The figure shows three views and two pictorial views of one solid part (mm, origin at its lowest corner). Answer the questions. Round coordinates to 2 decimals unless told otherwise and drop trailing zeros. Write each loop counter-clockwise with the first axis right and the second up, starting at its lowest first coordinate (ties: lowest second). Pieces come first, ordered by that corner, then holes. Notation, with made-up numbers: M -26,43 L 12,43 A20 cw 12,78 Z; hole C 38.5,42 d6. An arc over 180 degrees is marked long. Answer in a Markdown table with one row per item.
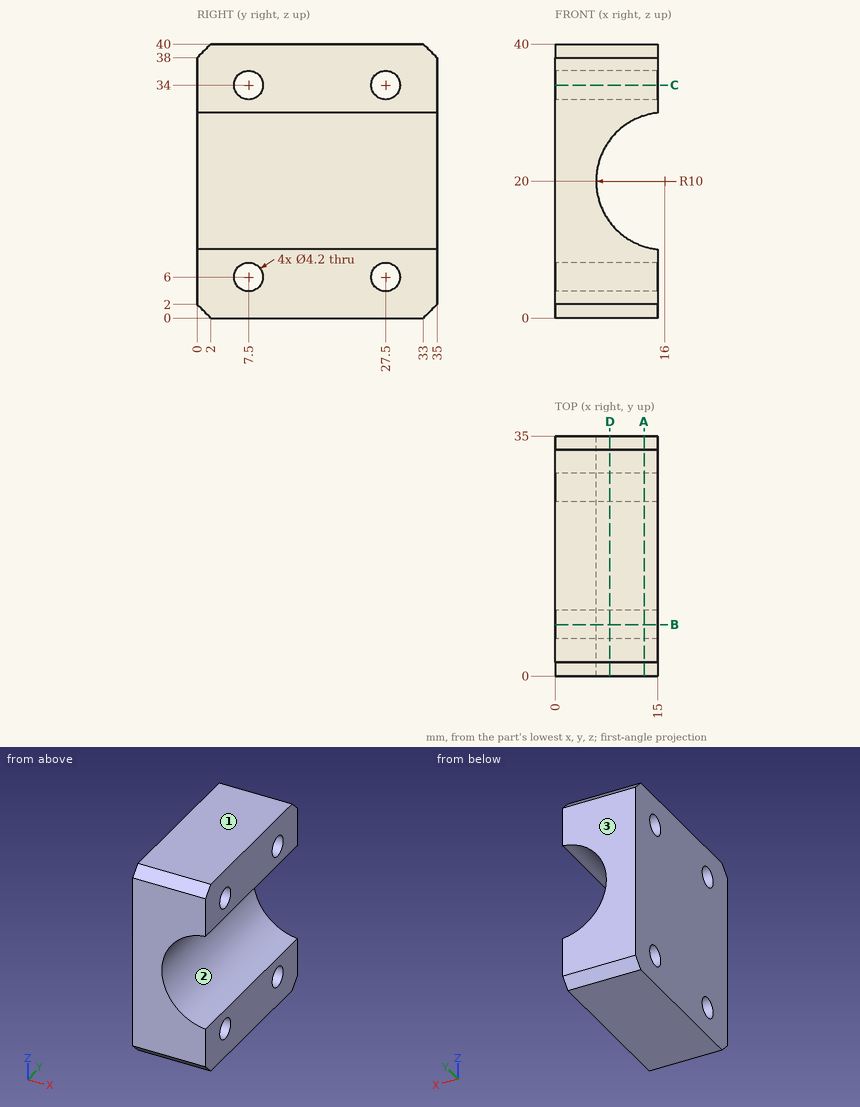
1. Given pin 1 (2 mm diameter, centred on y = 18, z = 26, fed in from +X), flat-ended and moving along its own axis, determine where the tip first touches the part or whether it passes through.
Calculated:
| item | result |
|---|---|
| pin 1 | stops at x = 8.86 |
2. The part is cut by section B-B (y = 7.5). Determine the outline of the cut face in (x, z), plus the area to 3 significant figures.
Calculated:
| item | result |
|---|---|
| outline | M 0,0 L 15,0 L 15,3.9 L 0,3.9 Z; M 0,8.1 L 15,8.1 L 15,10.05 A10 cw 15,29.95 L 15,31.9 L 0,31.9 Z; M 0,36.1 L 15,36.1 L 15,40 L 0,40 Z |
| area | 337 mm² |
3. The part is cut by section D-D (x = 8). Determine the outline of the cut face in (y, z), plus the area to 3 significant figures.
Calculated:
| item | result |
|---|---|
| outline | M 0,2 L 2,0 L 33,0 L 35,2 L 35,14 L 0,14 Z; M 0,26 L 35,26 L 35,38 L 33,40 L 2,40 L 0,38 Z; hole C 7.5,6 d4.2; hole C 7.5,34 d4.2; hole C 27.5,6 d4.2; hole C 27.5,34 d4.2 |
| area | 917 mm² |
4. Consider line 1 along Y through (x, z) = (9.75, 34); line 2 along Y through (x, z) = (10.75, 7); line 3 along Z through (x, y) = (4.75, 6.5). Determine where each line is inside the solid, lowest interval first. Write a range as from..to.
Calculated:
| item | result |
|---|---|
| line 1 | y = 0..5.4, 9.6..25.4, 29.6..35 |
| line 2 | y = 0..5.65, 9.35..25.65, 29.35..35 |
| line 3 | z = 0..4.15, 7.85..32.15, 35.85..40 |
5. The part is cut by section A-A (x = 13). Determine the outline of the cut face in (y, z), plus the area to 3 significant figures.
Calculated:
| item | result |
|---|---|
| outline | M 0,2 L 2,0 L 33,0 L 35,2 L 35,10.46 L 0,10.46 Z; M 0,29.54 L 35,29.54 L 35,38 L 33,40 L 2,40 L 0,38 Z; hole C 7.5,6 d4.2; hole C 7.5,34 d4.2; hole C 27.5,6 d4.2; hole C 27.5,34 d4.2 |
| area | 669 mm² |
6. The part is cut by section C-C (z = 34). Determine the outline of the cut face in (x, y).
Calculated:
| item | result |
|---|---|
| outline | M 0,0 L 15,0 L 15,5.4 L 0,5.4 Z; M 0,9.6 L 15,9.6 L 15,25.4 L 0,25.4 Z; M 0,29.6 L 15,29.6 L 15,35 L 0,35 Z |
7. Determine the mould class of the marked faces 1, 2 and 3 for opening direction Z: released by +Z, released by -Z, zero draft, split by the parting line, or undercut.
Calculated:
| item | result |
|---|---|
| face 1 | released by +Z |
| face 2 | undercut |
| face 3 | zero draft |
